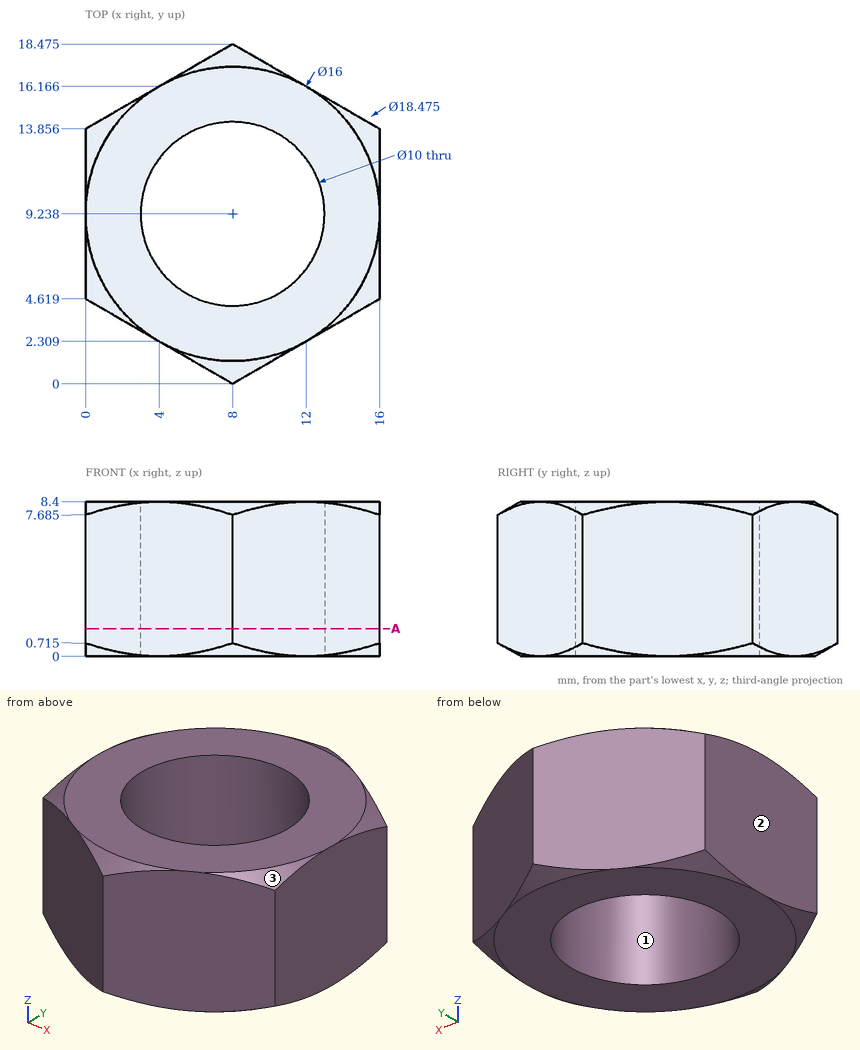
Could you check a few things on this drawing? It's one solid part, dimensions in mm from its lowest x, y, z. Coordinates: 2 decimals unless noted, no trailing zeros. Write each loop counter-clockwise with the first axis right and the second up, starting at its lowest first coordinate (ties: lowest second). Pieces come first, ordered by that corner, then holes. Notation, with made-up numbers: (-10, 7) - (41, 7) arc R21 cw to (41, 18) - close; hole circle Ø2 at (15, 68.25). An arc over 180 degrees is marked (long way). Put each result on its own line as item: value. Start each with the question number.
Q1. Thinking about a two-plate mould opening in X: for the marked faces 1, 2 and 3, which applies, pulls with the +X half, pulls with the -X half, needs draft (parallel to the pull), parting line crosses it, or undercut?
Q2. I want a section at A-A on z = 1.5. Write out the boundary of the cut face in (x, y) (1 decimal).
Q3. Please list where these lines run through material, in increasing order: L1, parallel to X at y = 10.5, z = 5.25; L2, parallel to Y at x = 9.5, z = 1.5 (1 decimal); L3, parallel to X at y = 6.25, z = 0.5.
Q4. I'm going to push flat-ended pins straight in: P1, Ø1, axis at x = 9.5, y = 3, coming from the -Z side; P2, Ø1, axis at x = 4.5, z = 2.5, coming from the -Y side; P3, Ø1, axis at y = 14.5, z = 4.5, coming from the -X side; P4, Ø4, axis at y = 16, z = 7.5, coming from the +X side. Where does each tip first touch, or does it pass through?
Checks:
1. face 1: undercut
1. face 2: pulls with the -X half
1. face 3: pulls with the +X half
2. outline: (0, 4.6) - (8, 0) - (16, 4.6) - (16, 13.9) - (8, 18.5) - (0, 13.9) - close; hole circle Ø10 at (8, 9.2)
3. L1: 0 to 3.16, 12.84 to 16
3. L2: 0.9 to 4.5, 14 to 17.6
3. L3: 0 to 3.99, 12.01 to 16
4. P1: z = 0
4. P2: y = 1.73
4. P3: x = 0.25
4. P4: x = 15.75
